Part model, mm, in its own coordinate system. Give positions to 0.01 mm unless a question says otherwise; leave off trailing zeros. Order: outer loops, then holes, each group sorted by start corner. A loop starts at its lowest first (then second) coordinate and runs counter-clockwise, first axis right, second up. Notation, with made-up numbers: (85.5, 74) - (139.5, 74) arc R17 cw to (139.5, 84) - close; hole circle Ø10 at (48.25, 84). An arc over 180 degrees is marked (long way). One line per item, written item: value.
```python
from build123d import *

# Parameters (mm, degrees)
BOSS_EXTRUDE1_DEPTH = 435
SKETCH2_R           = 8.5
CUT_EXTRUDE1_DEPTH  = 435
CUT_EXTRUDE2_DEPTH  = 435
SKETCH4_R           = 4.25
CUT_EXTRUDE3_DEPTH  = 435


with BuildPart() as part:
    # Sketch1 → Boss-Extrude1 (new body)
    with BuildSketch(Plane.XY):
        with BuildLine():
            Line((0, 0), (-30, 0))
            Line((-30, 0), (-30, -60))
            Line((-30, -60), (0, -60))
            Line((0, -60), (0, -58.715972734))
            ThreePointArc((0, -58.715972734), (-0.735871259, -56.747795647), (-2.582480697, -55.745168528))
            Line((-2.582480697, -55.745168528), (-18.835038606, -53.461020473))
            ThreePointArc((-18.835038606, -53.461020473), (-22.528257481, -51.455766235), (-24, -47.519412061))
            Line((-24, -47.519412061), (-24, -12.480587939))
            ThreePointArc((-24, -12.480587939), (-22.528257481, -8.544233765), (-18.835038606, -6.538979527))
            Line((-18.835038606, -6.538979527), (-2.582480697, -4.254831472))
            ThreePointArc((-2.582480697, -4.254831472), (-0.735871259, -3.252204353), (0, -1.284027266))
            Line((0, -1.284027266), (0, 0))
        make_face()
    extrude(amount=BOSS_EXTRUDE1_DEPTH)

    # Sketch2 → Cut-Extrude1 (cut)
    with BuildSketch(Plane.ZY.offset(30)):
        with Locations(Location((35.5, -30, 0), (0, 0, 270))):
            Circle(SKETCH2_R)
    extrude(amount=-CUT_EXTRUDE1_DEPTH, mode=Mode.SUBTRACT)

    # Sketch3 → Cut-Extrude2 (cut)
    with BuildSketch(Plane(origin=(0, 0, 0), x_dir=(1, 0, 0), z_dir=(0, 1, 0))):
        Polygon((-15, 0), (0, 0), (0, -35), align=None)
    extrude(amount=-CUT_EXTRUDE2_DEPTH, mode=Mode.SUBTRACT)

    # Sketch4 → Cut-Extrude3 (cut)
    with BuildSketch(Plane.ZY.offset(30)):
        with Locations(Location((95, -30, 0), (0, 0, 270))):
            Circle(SKETCH4_R)
        with Locations(Location((146, -30, 0), (0, 0, 270))):
            Circle(SKETCH4_R)
    extrude(amount=-CUT_EXTRUDE3_DEPTH, mode=Mode.SUBTRACT)


solid = part.part
```
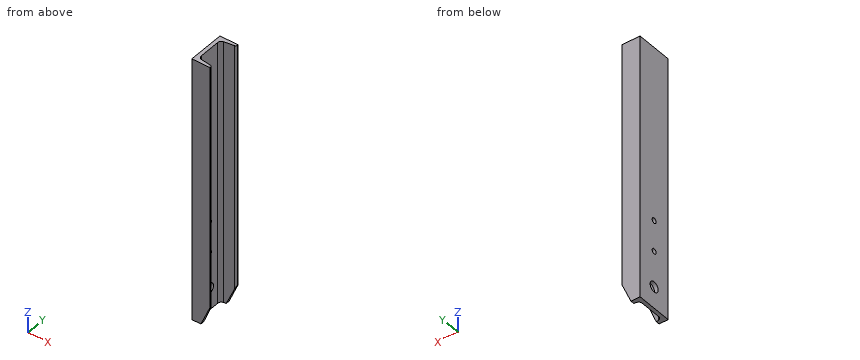
1) Drop flat-ended pins along their axis: P1, Ø10, axis at y = -32.5, z = 294.5, coming from the +X side; P2, Ø7.5, axis at y = -30, z = 95, coming from the +X side. Give the stop position or say it passes through.
Answer:
P1: stops at x = -24
P2: passes through
2) Slice it at A-A on y = -30. Write the cut outline in (x, z).
Answer:
outline: (-30, 0) - (-24, 0) - (-24, 27) - (-30, 27) - close; (-30, 44) - (-24, 44) - (-24, 90.75) - (-30, 90.75) - close; (-30, 99.25) - (-24, 99.25) - (-24, 141.75) - (-30, 141.75) - close; (-30, 150.25) - (-24, 150.25) - (-24, 435) - (-30, 435) - close
3) Wall check: line 1 along Z through (x, y) = (-25.75, -30); line 2 along X through (y, z) = (-15, 58); line 3 along Y through (x, z) = (-10.5, 167). Give the ranges that are in metal, low to high. Write a range as [from, to].
Answer:
line 1: z = [0, 27], [44, 90.75], [99.25, 141.75], [150.25, 435]
line 2: x = [-30, -24]
line 3: y = [-60, -54.63], [-5.37, 0]
4) Slice it at C-C on z = 95. Write the cut outline in (x, y).
Answer:
outline: (-30, -60) - (0, -60) - (0, -58.72) arc R3 ccw to (-2.58, -55.75) - (-18.84, -53.46) arc R6 cw to (-24, -47.52) - (-24, -34.25) - (-30, -34.25) - close; (-30, -25.75) - (-24, -25.75) - (-24, -12.48) arc R6 cw to (-18.84, -6.54) - (-2.58, -4.25) arc R3 ccw to (0, -1.28) - (0, 0) - (-30, 0) - close
5) Slice it at D-D on z = 314. Write the cut outline in (x, y), then the cut area to 3 significant figures.
Answer:
outline: (-30, -60) - (0, -60) - (0, -58.72) arc R3 ccw to (-2.58, -55.75) - (-18.84, -53.46) arc R6 cw to (-24, -47.52) - (-24, -12.48) arc R6 cw to (-18.84, -6.54) - (-2.58, -4.25) arc R3 ccw to (0, -1.28) - (0, 0) - (-30, 0) - close
area: 636 mm2
6) Slice it at B-B on x = -6.25. Write the cut outline in (y, z).
Answer:
outline: (-60, 20.42) - (-55.23, 20.42) - (-55.23, 435) - (-60, 435) - close; (-4.77, 20.42) - (0, 20.42) - (0, 435) - (-4.77, 435) - close
